Source: three-view drawing plus pictorial views. Frame: mm from the lowest corner of the part. Round coordinates to 2 decimals unless told otherwise and drop trailing zeros. Loops run counter-clockwise (first coordinate to the right, second up) from the corner with the lowest first, then second, coordinate; pieces in that order, holes last. Notation, with made-up numbers: M 37.25,23 L 41.25,23 A32 ccw 41.25,60 Z; hole C 10,-6 d8. An arc over 180 degrees is marked long. Write each question's results on one line, items separated by ' | '.
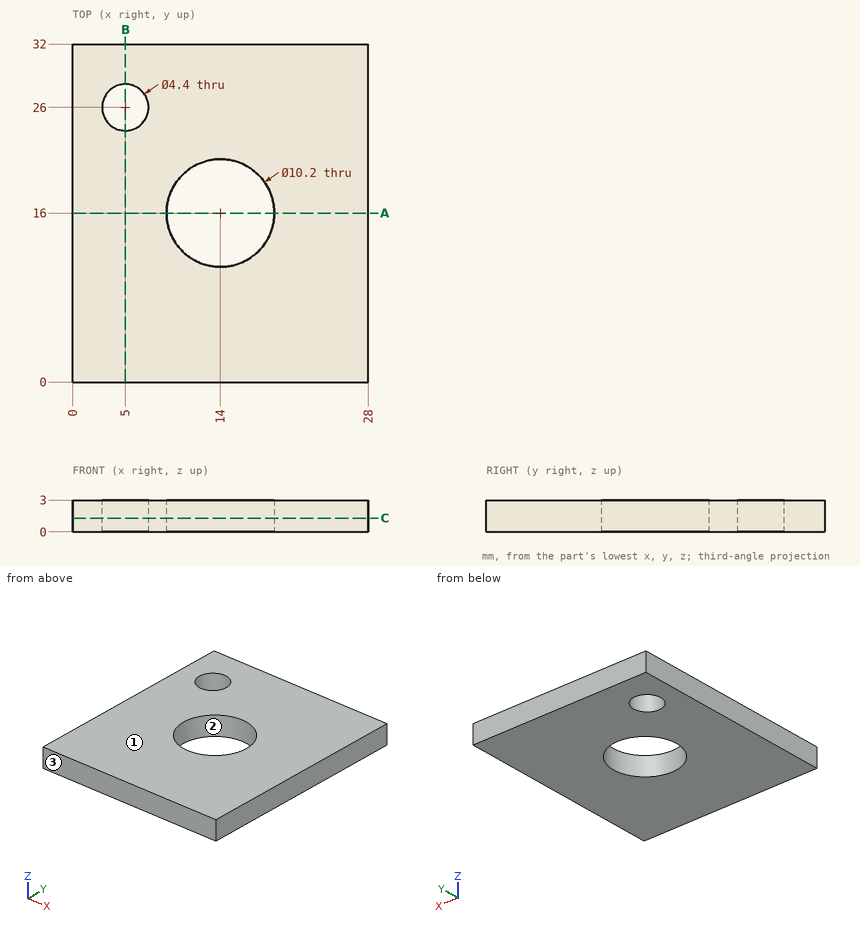
1. Section A-A (y = 16). Output: boundary loops of the cut face in (x, z).
Answer key:
outline: M 0,0 L 8.9,0 L 8.9,3 L 0,3 Z; M 19.1,0 L 28,0 L 28,3 L 19.1,3 Z
2. Section C-C (z = 1.3). Output: boundary loops of the cut face in (x, y), then the cut area to 3 significant figures.
Answer key:
outline: M 0,0 L 28,0 L 28,32 L 0,32 Z; hole C 5,26 d4.4; hole C 14,16 d10.2 | area: 799 mm²
3. Draft query along Y for the marked faces 1, 2 and 3. Return one class per face: pulls with the +Y half, pulls with the -Y half, needs draft (parallel to the pull), parting line crosses it, or undercut.
Answer key:
face 1: needs draft | face 2: undercut | face 3: pulls with the -Y half
4. Section B-B (x = 5). Output: boundary loops of the cut face in (y, z).
Answer key:
outline: M 0,0 L 23.8,0 L 23.8,3 L 0,3 Z; M 28.2,0 L 32,0 L 32,3 L 28.2,3 Z
5. Ray query, probe 1 along X at (y, z) = (16, 0.85); probe 2 along Y at (x, z) = (5, 2.05); probe 3 along Y at (x, z) = (18.25, 1.85). Return the intervals inside material, ascending.
Answer key:
probe 1: x = 0 to 8.9, 19.1 to 28 | probe 2: y = 0 to 23.8, 28.2 to 32 | probe 3: y = 0 to 13.18, 18.82 to 32
6. Pin query (flat end, axial travel): P1, Ø1.5, axis at x = 4.5, z = 1.5, coming from the -Y side. Return the tip coordinate at first contact, or that it passes through.
Answer key:
P1: stops at y = 0
